The figure shows three views and two pictorial views of one solid part (mm, origin at its lowest corner). Answer the questions. A direction names the side the tool comes from. Give positions to 0.01 mm unless a question says otherwise; leave off trailing zeros. Order: outer loops, then holes, each group sorted by start corner. A loop starts at its lowest first (then second) coordinate and runs counter-clockwise, first axis right, second up. Notation, with made-up numbers: (84.25, 46) - (139.25, 46) arc R34 ccw to (139.25, 77) - close; hole circle Ø10 at (46, 6). An arc over 180 degrees is marked (long way). Answer as a JSON object with one key per item and string values. Group by question number.
Q1. Consider line 1 (X direction, y = 140, z = 70); line 2 (Y direction, x = 85, z = 19). Determine where each line is inside the solid, lowest interval first.
Q2. A cutting plane is placed at A-A, the plane y = 113.5. Give the vertices of the cut face in (x, z).
Q3. Given pin 1 (10 mm diameter, centred on y = 66, z = 131, fed in from -X), flat-ended and moving along its own axis, determine where the tip first touches the part or whether it passes through.
Q4. A cutting plane is placed at C-C, the plane x = 93.5. Give the vertices of the cut face in (y, z), and give its area (3 significant figures).
Q5. For the marked faces 1 and 2, determine the directions among +Z, -Z, +X, -X, +Y, -Y from which every point of the face is accessible in a straight line to the end or side of a thin tool.
Q6. A cutting plane is placed at B-B, the plane z = 152. Give the vertices of the cut face in (x, y), and give its area (4 significant figures).
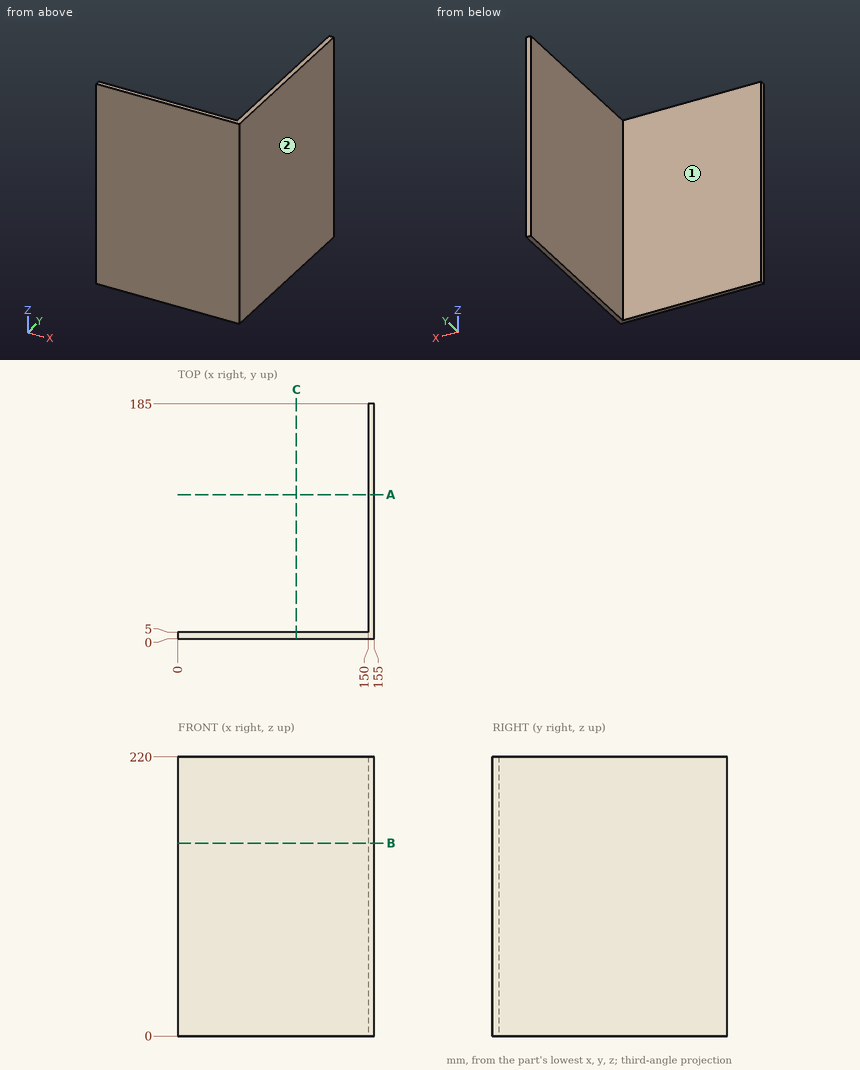
Reply:
{
 "1": {"line 1": "x = 150 to 155", "line 2": "y = 0 to 5"},
 "2": {"outline": "(150, 0) - (155, 0) - (155, 220) - (150, 220) - close"},
 "3": {"pin 1": "stops at x = 150"},
 "4": {"outline": "(0, 0) - (5, 0) - (5, 220) - (0, 220) - close", "area": "1,100 mm^2"},
 "5": {"face 1": "+Z, -Z, -X, +Y", "face 2": "+Z, -Z, +X, +Y, -Y"},
 "6": {"outline": "(0, 0) - (155, 0) - (155, 185) - (150, 185) - (150, 5) - (0, 5) - close", "area": "1,675 mm^2"}
}
